Check sheet for the modelled part. Datum: model origin and axes. Units: mm. Coordinates: 2 decimals unless noted, no trailing zeros. Loops run counter-clockwise (first coordinate to the right, second up) from the corner with the lowest first, then second, coordinate; pieces in that order, holes last. Notation, with made-up numbers: M 50.25,2.5 L 87.25,2.5 A20 cw 87.25,6.5 Z; hole C -32,9.25 d8. An arc over 180 degrees is marked long. Use CSV: the item, a comma, the result in double quotes. Start each with the question number.
(1) Go/stop test with a flat-tipped pin: pin 1 Ø2 at (y, z) = (82, -1) entering from +X. Record where the tip stops, or that it passes through.
(2) Section check B-B on z = 2.5. Record the cut outline in (x, y).
(3) Section check A-A on y = 86. Record the cut outline in (x, z), and give its area (3 significant figures).
(4) Scan lines: line 1 (X direction, y = 142, z = 4); line 2 (X direction, y = 18.5, z = 1); line 3 (Y direction, x = 8.5, z = 1). Record each from-to range of solid material in increasing order.
(5) Section check C-C on x = 12. Record the cut outline in (y, z).
from build123d import *

# Parameters (mm, degrees)
BOSS_EXTRUDE1_DEPTH = 5
CHAMFER1_SIZE       = 20


with BuildPart() as part:
    # Sketch1 → Boss-Extrude1 (new, symmetric)
    with BuildSketch(Plane.XY):
        Polygon((0, 0), (65, 0), (65, 20), (20, 240), (0, 240), align=None)
    extrude(amount=BOSS_EXTRUDE1_DEPTH, both=True)

    # Chamfer1
    chamfer1_edges = [part.edges().sort_by_distance(p)[0] for p in [
        (0, 0, 0),
    ]]
    chamfer(chamfer1_edges, length=CHAMFER1_SIZE)


solid = part.part
Outcome:
1,pin 1,"stops at x = 52.52"
2,outline,"M 0,20 L 20,0 L 65,0 L 65,20 L 20,240 L 0,240 Z"
3,outline,"M 0,-5 L 51.5,-5 L 51.5,5 L 0,5 Z"
3,area,"515 mm²"
4,line 1,"x = 0 to 40.05"
4,line 2,"x = 1.5 to 65"
4,line 3,"y = 11.5 to 240"
5,outline,"M 8,-5 L 240,-5 L 240,5 L 8,5 Z"
